from build123d import *

# Parameters (mm, degrees)
BASE_PLATE_SKETCH_W             = 50
BASE_PLATE_SKETCH_H             = 170
BASE_PLATE_170X50X20_DEPTH      = 20
CLAMP_SADDLE_DEPTH              = 25
SADDLE_FILLET_R15_R             = 15
SADDLE_TO_PLATE_FILLET_R5_R     = 5
CLAMP_BOLT_HOLES_SKETCH_R       = 7.5
CLAMP_BOLT_HOLES_2X_15_DEPTH    = 25
MOUNTING_HOLES_SKETCH_R         = 7.5
MOUNTING_HOLES_2X_15_DEPTH      = 25
MOUNTING_START                  = 5
MOUNTING_HOLE_BOSSES_SKETCH_R   = 12.5
MOUNTING_HOLE_BOSSES_SKETCH_R_2 = 7.5
MOUNTING_HOLE_BOSSES_25_DEPTH   = 5
HOLE_BOSS_FILLET_R2_R           = 2
BASE_PLATE_CORNER_FILLETS_R15_R = 15
SUPPORT_RIB_DEPTH               = 17.5
SUPPORT_RIB_FILLET_R25_R        = 25
RIB_TO_PLATE_FILLET_R5_R        = 5


with BuildPart() as part:
    # Base Plate Sketch → Base Plate 170x50x20 (new body)
    with BuildSketch(Plane.XY):
        Rectangle(BASE_PLATE_SKETCH_W, BASE_PLATE_SKETCH_H)
    extrude(amount=BASE_PLATE_170X50X20_DEPTH)

    # Clamp Saddle Sketch → Clamp Saddle (add, symmetric)
    with BuildSketch(Plane(origin=(0, 0, 0), x_dir=(0, 0, -1), z_dir=(1, 0, 0))):
        with BuildLine():
            Line((-159.934479129, 25.889967638), (-179.934479129, 25.889967638))
            Line((-179.934479129, 25.889967638), (-229.717625742, 25.889967638))
            Line((-229.717625742, 25.889967638), (-229.717625742, 10.889967638))
            Line((-229.717625742, 10.889967638), (-178.029229322, 10.889967638))
            ThreePointArc((-178.029229322, 10.889967638), (-119.934479129, -34.110032362), (-61.839728936, 10.889967638))
            Line((-61.839728936, 10.889967638), (-20, 10.889967638))
            Line((-20, 10.889967638), (-20, 25.889967638))
            Line((-20, 25.889967638), (-79.934479129, 25.889967638))
            ThreePointArc((-79.934479129, 25.889967638), (-119.934479129, -14.110032362), (-159.934479129, 25.889967638))
        make_face()
    extrude(amount=CLAMP_SADDLE_DEPTH, both=True)

    # Saddle Fillet R15
    saddle_fillet_r15_edges = [part.edges().sort_by_distance(p)[0] for p in [
        (25, 18.389967638, 229.717625742),
        (-25, 18.389967638, 229.717625742),
    ]]
    fillet(saddle_fillet_r15_edges, radius=SADDLE_FILLET_R15_R)

    # Saddle To Plate Fillet R5
    saddle_to_plate_fillet_r5_edges = [part.edges().sort_by_distance(p)[0] for p in [
        (0, 25.889967638, 20),
    ]]
    fillet(saddle_to_plate_fillet_r5_edges, radius=SADDLE_TO_PLATE_FILLET_R5_R)

    # Clamp Bolt Holes Sketch → Clamp Bolt Holes 2xØ15 (cut, symmetric)
    with BuildSketch(Plane(origin=(0, 25.889967638, 0), x_dir=(1, 0, 0), z_dir=(0, 1, 0))):
        with Locations(Location((0, -46.822731441, 0), (0, 0, 270))):
            Circle(CLAMP_BOLT_HOLES_SKETCH_R)
        with Locations(Location((0, -196.822731441, 0), (0, 0, 90))):
            Circle(CLAMP_BOLT_HOLES_SKETCH_R)
    extrude(amount=CLAMP_BOLT_HOLES_2X_15_DEPTH, both=True, mode=Mode.SUBTRACT)

    # Mounting Holes Sketch → Mounting Holes 2xØ15 (cut, symmetric)
    with BuildSketch(Plane.XY.offset(20)):
        with Locations((0, 63.122206812)):
            Circle(MOUNTING_HOLES_SKETCH_R)
        with Locations((0, -63.861920173)):
            Circle(MOUNTING_HOLES_SKETCH_R)
    extrude(amount=MOUNTING_HOLES_2X_15_DEPTH, both=True, mode=Mode.SUBTRACT)

    # Mounting Hole Bosses Sketch → Mounting Hole Bosses Ø25 (add)
    # profile 1 of 2: a face of its own
    with BuildSketch(Plane.XY.offset(20).offset(MOUNTING_START)):
        with Locations((0, 63.122206812)):
            Circle(MOUNTING_HOLE_BOSSES_SKETCH_R)
        with Locations((0, 63.122206812)):
            Circle(MOUNTING_HOLE_BOSSES_SKETCH_R_2, mode=Mode.SUBTRACT)
    # profile 2 of 2: a face of its own
    with BuildSketch(Plane.XY.offset(20).offset(MOUNTING_START)):
        with Locations((0, -63.861920173)):
            Circle(MOUNTING_HOLE_BOSSES_SKETCH_R)
        with Locations((0, -63.861920173)):
            Circle(MOUNTING_HOLE_BOSSES_SKETCH_R_2, mode=Mode.SUBTRACT)
    extrude(amount=-MOUNTING_HOLE_BOSSES_25_DEPTH)

    # Hole Boss Fillet R2
    hole_boss_fillet_r2_edges = [part.edges().sort_by_distance(p)[0] for p in [
        (-12.5, 63.122206812, 25),
        (-12.5, -63.861920173, 25),
    ]]
    fillet(hole_boss_fillet_r2_edges, radius=HOLE_BOSS_FILLET_R2_R)

    # Base Plate Corner Fillets R15
    base_plate_corner_fillets_r15_edges = [part.edges().sort_by_distance(p)[0] for p in [
        (25, -85, 10),
        (-25, -85, 10),
        (-25, 85, 10),
        (25, 85, 10),
    ]]
    fillet(base_plate_corner_fillets_r15_edges, radius=BASE_PLATE_CORNER_FILLETS_R15_R)

    # Support Rib Sketch → Support Rib (add, symmetric)
    with BuildSketch(Plane(origin=(0, 0, 0), x_dir=(0, 0, -1), z_dir=(1, 0, 0))):
        with BuildLine():
            Line((-205.743047043, 10.889967638), (-205.743047043, -37.074588444))
            Line((-205.743047043, -37.074588444), (-20, -37.074588444))
            Line((-20, -37.074588444), (-20, 10.889967638))
            Line((-20, 10.889967638), (-61.839728936, 10.889967638))
            ThreePointArc((-61.839728936, 10.889967638), (-119.934479129, -34.110032362), (-178.029229322, 10.889967638))
            Line((-178.029229322, 10.889967638), (-205.743047043, 10.889967638))
        make_face()
    extrude(amount=SUPPORT_RIB_DEPTH, both=True)

    # Support Rib Fillet R25
    support_rib_fillet_r25_edges = [part.edges().sort_by_distance(p)[0] for p in [
        (0, -37.074588444, 205.743047043),
    ]]
    fillet(support_rib_fillet_r25_edges, radius=SUPPORT_RIB_FILLET_R25_R)

    # Rib To Plate Fillet R5
    rib_to_plate_fillet_r5_edges = [part.edges().sort_by_distance(p)[0] for p in [
        (0, -37.074588444, 20),
    ]]
    fillet(rib_to_plate_fillet_r5_edges, radius=RIB_TO_PLATE_FILLET_R5_R)


solid = part.part
Work out the finished part from the listing and answer in its coordinate system (mm). A direction names the side the tool comes from. Coordinates: 2 decimals unless noted, no trailing zeros. Loops run counter-clockwise (first coordinate to the right, second up) from the corner with the lowest first, then second, coordinate; pieces in that order, holes last. Notation, with made-up numbers: (-17.75, 78.25) -> (41.25, 78.25) arc R14 cw to (41.25, 89.25) -> close; hole circle Ø7 at (47.25, 34). An arc over 180 degrees is marked (long way). Write each question's results on one line, items separated by ' | '. Start each with the question number.
1) For faces 4 (the cylindrical face through (21.3, -34.1, 121)), 5 (the flat face through (-21, 10.89, 41)), 6 (the flat face through (0, -47, 20)), 7 (the cylindrical face through (-2.71, -76.065, 21.521)), 8 (the cylindrical face through (-0.33, 18.495, 204.315)), determine the directions among +Z, -Z, +X, -X, +Y, -Y from which every point of the face is accessible in a straight line to the end or side of a thin tool.
2) Find section A-A on y = 15. Determine the outline of the cut face in (x, z), then the cut area to 3 significant figures.
3) Flat-ended cylindrical pins translate along their axes: P1, Ø4, axis at x = 20.5, z = 40.5, coming from the -Y side; P2, Ø1, axis at y = -5.5, z = 51, coming from the -X side; P3, Ø11.5, axis at x = -2.5, y = -1, coming from the +Z side. Find the tip coordinate at first contact, or state that the pin passes through.
4) Find section D-D on x = 0. Count the separate pieces of the cut face and the enclosed holes in it, then the cut area to 3 significant figures.
5) The mould has two halves that part along Z. Classify faces 1 (the cylindrical face through (-21.2, -34.1, 121)), 2 (the cylindrical face through (0.25, -29.56, 198.61)), 3 (the cylindrical face through (-20.72, 80.49, 10.14)): pulls with the +Z half, pulls with the -Z half, needs draft (parallel to the pull), parting line crosses it, or undercut.
6) Find section C-C on x = 20. Determine the outline of the cut face in (y, z).
7) Find section B-B on z = 27.5. Determine the outline of the cut face in (x, y), then the cut area to 3 significant figures.
8) Consider line 1 along Y through (x, z) = (0, 7.75); line 2 along Z through (x, y) = (3.5, 23); line 3 along Z through (x, y) = (22.5, 9). Determine where each line is inside the solid, lowest interval first.
Response values:
1) face 4: +X, -Y | face 5: -X, -Y | face 6: none | face 7: +Z | face 8: +Y
2) outline: (-25, 0) -> (25, 0) -> (25, 81.45) -> (-25, 81.45) -> close; (-25, 158.42) -> (25, 158.42) -> (25, 214.72) arc R15 ccw to (10, 229.72) -> (-10, 229.72) arc R15 ccw to (-25, 214.72) -> close; hole circle Ø15 at (0, 46.82); hole circle Ø15 at (0, 196.82) | area: 7,190 mm^2
3) P1: stops at y = 10.89 | P2: stops at x = -17.5 | P3: stops at z = 205.74
4) separate pieces: 3 | enclosed holes: 0 | area: 11,900 mm^2
5) face 1: undercut | face 2: pulls with the +Z half | face 3: needs draft
6) outline: (-81.18, 0) -> (81.18, 0) -> (81.18, 20) -> (30.89, 20) arc R5 cw to (25.89, 25) -> (25.89, 79.93) arc R40 cw to (25.89, 159.93) -> (25.89, 225.9) -> (10.89, 225.9) -> (10.89, 178.03) arc R60 ccw to (10.89, 61.84) -> (10.89, 20) -> (-81.18, 20) -> close
7) outline: (-25, 10.89) -> (-17.5, 10.89) -> (-17.5, -37.07) -> (17.5, -37.07) -> (17.5, 10.89) -> (25, 10.89) -> (25, 25.89) -> (-25, 25.89) -> close | area: 2,430 mm^2
8) line 1: y = -85 to -71.36, -56.36 to 55.62, 70.62 to 85 | line 2: z = 0 to 40.19, 53.46 to 80.04, 159.83 to 190.19, 203.46 to 229.72 | line 3: z = 0 to 20, 62.36 to 83.68, 156.19 to 177.51
